from build123d import *

# Parameters (mm, degrees)
EXTRUDE_1_DEPTH = 15


with BuildPart() as part:
    # 草图2 → 拉伸-薄壁1 (new, symmetric)
    with BuildSketch(Plane(origin=(0, 0, 0), x_dir=(0, 0, -1), z_dir=(1, 0, 0))):
        with BuildLine():
            Line((-1496.41, -51.25), (0, -51.25))
            ThreePointArc((0, -51.25), (51.25, 0), (0, 51.25))
            Line((0, 51.25), (-1496.41, 51.25))
            ThreePointArc((-1496.41, 51.25), (-1547.66, 0), (-1496.41, -51.25))
        make_face()
        with BuildLine():
            Line((-1496.41, -46.75), (0, -46.75))
            ThreePointArc((0, -46.75), (46.75, 0), (0, 46.75))
            Line((0, 46.75), (-1496.41, 46.75))
            ThreePointArc((-1496.41, 46.75), (-1543.16, 0), (-1496.41, -46.75))
        make_face(mode=Mode.SUBTRACT)
    extrude(amount=EXTRUDE_1_DEPTH, both=True)


solid = part.part
The model under review builds one solid part; all positions refer to its coordinate system, in mm. A direction names the side the tool comes from. Give positions to 0.01 mm unless a question says otherwise; leave off trailing zeros. Order: outer loops, then holes, each group sorted by start corner. A loop starts at its lowest first (then second) coordinate and runs counter-clockwise, first axis right, second up. Notation, with made-up numbers: (8, 24) -> (59, 24) arc R20 ccw to (59, 41) -> close; hole circle Ø6 at (51, 41). An arc over 180 degrees is marked (long way). Write item = value, one per line. Start each with the question number.
(1) Tool access review of faces 4 (the flat face through (0, 46.75, 738)), 5 (the flat face through (0, 51.25, 738)): name each direction out of +Z, -Z, +X, -X, +Y, -Y from which nothing blocks a thin tool from reaching the whole face with its end or side.
(2) For L1, parallel to Y at x = 3.25, z = 789.5; L2, parallel to Z at x = -7.5, y = 10.5; L3, parallel to Z at x = 11.75, y = 41.5, list the stretches that pass through material, from the lowest coordinate up. Write a range as from..to.
(3) For pin 1 Ø5 at (x, y) = (-7, -2.5) entering from -Z; pin 2 Ø10 at (x, y) = (-4.5, 26.5) entering from +Z, all flat-tipped, find the tip position at first contact; note any pin that passes through.
(4) Take a section at B-B (y = 0). Write out the cut boundary in (x, z), plus the area to 3 significant figures.
(5) Take a section at A-A (z = 685). Write out the cut boundary in (x, y), plus the area to 3 significant figures.
(6) Draft analysis for pull direction Z (two halves, no side actions). For faces 1 (the flat face through (0, -51.25, 759)), 2 (the cylindrical face through (0.21, 1.127, 1547.648)), 3 (the flat face through (0, -46.75, 759)), state which applies: +Z half, -Z half, draft (parallel to the pull), parting line (faces both ways), or undercut.
Returned:
q1.face_4 = +X, -X
q1.face_5 = +Z, -Z, +X, -X, +Y
q2.L1 = -51.25..-46.75, 46.75..51.25
q2.L2 = -50.16..-45.56, 1541.97..1546.57
q2.L3 = -30.07..-21.52, 1517.93..1526.48
q3.pin_1 = -51.25
q3.pin_2 = 1542.93
q4.outline = (-15, -51.25) -> (15, -51.25) -> (15, -46.75) -> (-15, -46.75) -> close; (-15, 1543.16) -> (15, 1543.16) -> (15, 1547.66) -> (-15, 1547.66) -> close
q4.area = 270 mm²
q5.outline = (-15, -51.25) -> (15, -51.25) -> (15, -46.75) -> (-15, -46.75) -> close; (-15, 46.75) -> (15, 46.75) -> (15, 51.25) -> (-15, 51.25) -> close
q5.area = 270 mm²
q6.face_1 = draft
q6.face_2 = +Z half
q6.face_3 = undercut
